Could you check a few things on this model? Use its own coordinates, in mm. A direction names the side the tool comes from. Round coordinates to 2 decimals unless told otherwise and drop trailing zeros. Write each loop counter-clockwise with the first axis right and the second up, starting at its lowest first coordinate (ties: lowest second). Pieces come first, ordered by that corner, then holes. Notation, with made-up numbers: (75.25, 3.5) - (84.25, 3.5) arc R23 cw to (84.25, 22.5) - close; hole circle Ø7 at (-10, 9.25). An arc over 180 degrees is marked (long way). Put each result on its own line as item: value.
from build123d import *

# Parameters (mm, degrees)
SKETCH1_R           = 40
SKETCH1_R_2         = 4
BOSS_EXTRUDE1_DEPTH = 7
CHAMFER1_SIZE       = 0.5


with BuildPart() as part:
    # Sketch1 → Boss-Extrude1 (new, symmetric)
    with BuildSketch(Plane.XY):
        Circle(SKETCH1_R)
        Circle(SKETCH1_R_2, mode=Mode.SUBTRACT)
    extrude(amount=BOSS_EXTRUDE1_DEPTH, both=True)

    # Sketch2 → Cut-Revolve1 (revolve, cut)
    with BuildSketch(Plane(origin=(0, 0, 0), x_dir=(0, 0, -1), z_dir=(1, 0, 0)), mode=Mode.PRIVATE) as cut_revolve1_sk:
        Polygon((-5, 39.744407704), (-2.448600638, 35.325254378), (2.448600638, 35.325254378), (5, 39.744407704), (5, 40), (-5, 40), align=None)
    revolve(cut_revolve1_sk.sketch.rotate(Axis((0, 0, 7), (0, 0, -1)), 90), axis=Axis((0, 0, 7), (0, 0, -1)), mode=Mode.SUBTRACT)

    # Chamfer1
    chamfer1_edges = [part.edges().sort_by_distance(p)[0] for p in [
        (-4, 0, -7),
        (-4, 0, 7),
    ]]
    chamfer(chamfer1_edges, length=CHAMFER1_SIZE)


solid = part.part
(1) If we mould it in two halves opening along X, with no side actions, what happens to faces 1 (the face through (33.899, -10.675, 2.572)), 2 (the face through (8, 1, 7)), 3 (the face through (-0.867, -3.905, -0.091))? For each: pulls with the +X half, pulls with the -X half, needs draft (parallel to the pull), parting line crosses it, or undercut.
Values found:
face 1: parting line crosses it
face 2: needs draft
face 3: undercut
(2) I'm going to push flat-ended pins straight in: pin 1 (1.5 mm diameter, centred on y = 4.5, z = -4.5, fed in from +X); pin 2 (1.5 mm diameter, centred on y = -17.5, z = 1.5, fed in from -X); pin 3 (3 mm diameter, centred on x = 31, y = 28.5, fed in from -Z); pin 4 (1.5 mm diameter, centred on x = 0.5, z = -5.5, fed in from +Y). Where does each tip first touch, or does it pass through?
Values found:
pin 1: stops at x = 39.81
pin 2: stops at x = -31.1
pin 3: passes through
pin 4: stops at y = 40
(3) Imagine slicing it at C-C, the plane z = 4. List the corners of the cut face in (x, y) for me.
Values found:
outline: circle Ø76.02 at (0, 0); hole circle Ø8 at (0, 0)
(4) Imagine slicing it at A-A, the plane y = 0. List the corners of the cut face in (x, z) for me.
Values found:
outline: (-40, -7) - (-4.5, -7) - (-4, -6.5) - (-4, 6.5) - (-4.5, 7) - (-40, 7) - (-40, 5) - (-39.74, 5) - (-35.33, 2.45) - (-35.33, -2.45) - (-39.74, -5) - (-40, -5) - close; (4, -6.5) - (4.5, -7) - (40, -7) - (40, -5) - (39.74, -5) - (35.33, -2.45) - (35.33, 2.45) - (39.74, 5) - (40, 5) - (40, 7) - (4.5, 7) - (4, 6.5) - close
(5) Please list where these lines run through material, in increasing order: probe 1 along Y at (x, z) = (0, 1); probe 2 along Z at (x, y) = (33, -21.5); probe 3 along Z at (x, y) = (30.5, -24.5). Write a range as from..to.
Values found:
probe 1: y = -35.33..-4, 4..35.33
probe 2: z = -7..-4.79, 4.79..7
probe 3: z = -7..-4.64, 4.64..7
(6) For faces 4 (the face through (33.96, -10.69, -2.61)), 5 (the face through (-8.67, -39.05, 6.01)), which set-ups out of +Z, -Z, +X, -X, +Y, -Y let a thin tool reach every point of the face, with its end or its side?
Values found:
face 4: none
face 5: +Z, -Z
